Can you work these out from the model? Positions are in its coordinate system, mm. Face numbers are marked on the shaded views. A direction names the side the tool comes from. Round coordinates to 2 decimals unless told otherwise and drop trailing zeros. Loops run counter-clockwise (first coordinate to the right, second up) from the corner with the lowest first, then second, coordinate; pieces in that order, holes last.
```python
from build123d import *

# Parameters (mm, degrees)
SKETCH1_R           = 2
BOSS_EXTRUDE1_DEPTH = 28
CHAMFER1_SIZE       = 0.5
SKETCH3_W           = 9.979897522
SKETCH3_H           = 2.201799933
CUT_EXTRUDE1_DEPTH  = 6


with BuildPart() as part:
    # Sketch1 → Boss-Extrude1 (new body)
    with BuildSketch(Plane.XY):
        Circle(SKETCH1_R)
    extrude(amount=BOSS_EXTRUDE1_DEPTH)

    # Chamfer1
    chamfer1_edges = [part.edges().sort_by_distance(p)[0] for p in [
        (-2, 0, 0),
        (-2, 0, 28),
    ]]
    chamfer(chamfer1_edges, length=CHAMFER1_SIZE)

    # Sketch3 → Cut-Extrude1 (cut)
    with BuildSketch(Plane.XY.offset(28)):
        with Locations((0.02893888, 2.800899967)):
            Rectangle(SKETCH3_W, SKETCH3_H)
    extrude(amount=-CUT_EXTRUDE1_DEPTH, mode=Mode.SUBTRACT)


solid = part.part
```
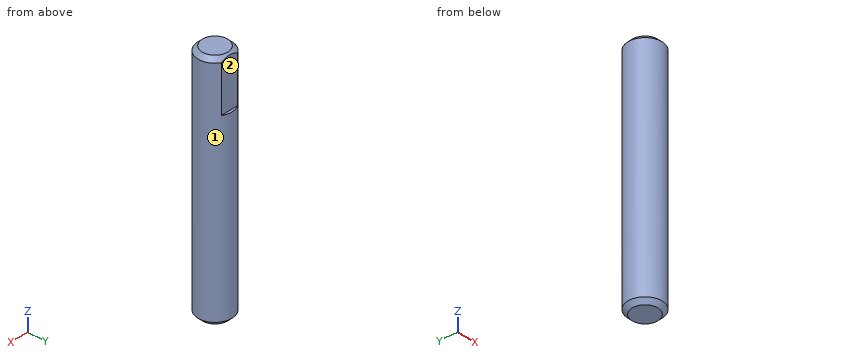
(1) Suppose I cut it at B-B (z = 5.25). Write out the boundary of the cut face in (x, y), then the cut area to 3 significant figures.
(2) If I drill on line 1 (X direction, y = -1.7, z = 22); line 2 (X direction, y = -0.1, z = 19), over which ranges is the centre line in solid material (lowest first)?
(3) Suppose I cut it at A-A (x = 0). Write out the boundary of the cut face in (y, z).
(4) Which directions (+Z, -Z, +X, -X, +Y, -Y) give clear straight access to the entire face, cutting with the end or side of a thin tool? Please do the marked faces 1 and 2.
(5) For pin 1 (1 mm diameter, centred on x = 1.5, y = 1.5, fed in from -Z); pin 2 (0.6 mm diameter, centred on x = 0.5, z = 23.5, fed in from +Y), each with a flat end and sliding along its axis, tell me the tip position at first contact or that it passes through.
Check result:
1. outline: circle Ø4 at (0, 0)
1. area: 12.6 mm2
2. line 1: x = -1.05 to 1.05
2. line 2: x = -2 to 2
3. outline: (-2, 0.5) - (-1.5, 0) - (1.5, 0) - (2, 0.5) - (2, 22) - (1.7, 22) - (1.7, 27.8) - (1.5, 28) - (-1.5, 28) - (-2, 27.5) - close
4. face 1: +Z, -Z
4. face 2: +Z, +X, -X, +Y
5. pin 1: stops at z = 0.12
5. pin 2: stops at y = 1.7
